For this review, use the dimensioned drawing (mm, ordinates from the lowest corner) and the shaded views. A direction names the side the tool comes from. Coordinates: 2 decimals unless noted, no trailing zeros. Loops run counter-clockwise (first coordinate to the right, second up) from the corner with the lowest first, then second, coordinate; pieces in that order, holes last. Notation, with made-up numbers: M -38.5,42 L 19.5,42 A23 cw 19.5,81 Z; hole C 0.25,16.5 d9. An arc over 180 degrees is marked long. Write item = value, one per line. Start each with the question number.
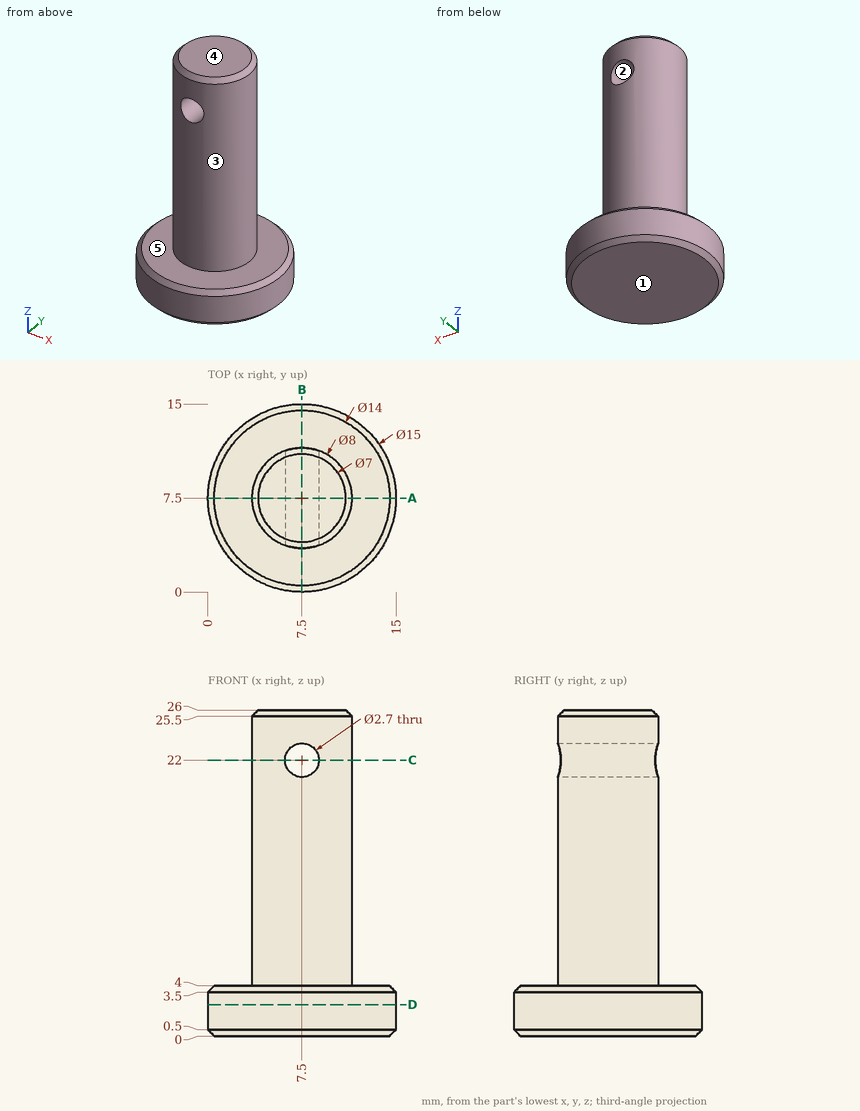
Q1. For the marked faces 4 and 5, list the 3-axis set-ups (+Z, -Z, +X, -X, +Y, -Y) from which the entire face can be reached by the end or side of a thin tool; tool diameter is ignored.
Q2. Add section D-D on z = 2.5. State the section outline as (x, y) points.
Q3. Clearance check with flat-ended pins moving along their axes: P1, Ø8, axis at x = 8, z = 21, coming from the -Y side; P2, Ø2, axis at y = 13.5, z = 15.5, coming from the -X side; P3, Ø4, axis at y = 6.5, z = 13, coming from the -X side; P4, Ø3, axis at x = 10.5, y = 5, coming from the -Z side. State where each tip first meets the part, or that it passes through.
Q4. To check wall thickness, follow line 1 (Z direction, x = 4.5, y = 3.75); line 2 (Z direction, x = 7.5, y = 9); line 3 (X direction, y = 7, z = 22). State the ranges of each line that lie inside material, in increasing order. Write a range as from..to.
Q5. Add section A-A on y = 7.5. State the section outline as (x, z) points.
Q6. Add section C-C on z = 22. State the section outline as (x, y) points, plus the area to 3 significant figures.
Q7. Add section B-B on x = 7.5. State the section outline as (y, z) points, plus the area to 3 significant figures.
Q8. Mouldability with a two-part tool opening along X and no side actions: class the marked faces 1, 2 and 3 as released by +X, released by -X, zero draft, split by the parting line, or undercut.
Values follow:
q1.face_4 = +Z, +X, -X, +Y, -Y
q1.face_5 = +Z
q2.outline = C 7.5,7.5 d15
q3.P1 = 3.5
q3.P2 = through
q3.P3 = 3.5
q3.P4 = 0
q4.line_1 = 0..4
q4.line_2 = 0..20.65, 23.35..26
q4.line_3 = 3.53..6.15, 8.85..11.47
q5.outline = M 0,0.5 L 0.5,0 L 14.5,0 L 15,0.5 L 15,3.5 L 14.5,4 L 11.5,4 L 11.5,25.5 L 11,26 L 4,26 L 3.5,25.5 L 3.5,4 L 0.5,4 L 0,3.5 Z; hole C 7.5,22 d2.7
q6.outline = M 6.15,3.73 L 6.15,11.27 A4 ccw Z; M 8.85,3.73 A4 ccw 8.85,11.27 Z
q6.area = 29.1 mm2
q7.outline = M 0,0.5 L 0.5,0 L 14.5,0 L 15,0.5 L 15,3.5 L 14.5,4 L 11.5,4 L 11.5,20.65 L 3.5,20.65 L 3.5,4 L 0.5,4 L 0,3.5 Z; M 3.5,23.35 L 11.5,23.35 L 11.5,25.5 L 11,26 L 4,26 L 3.5,25.5 Z
q7.area = 214 mm2
q8.face_1 = zero draft
q8.face_2 = undercut
q8.face_3 = split by the parting line
